Design review of the part built by this model. Coordinates are the model's own, in mm. A direction names the side the tool comes from. Coordinates: 2 decimals unless noted, no trailing zeros. Loops run counter-clockwise (first coordinate to the right, second up) from the corner with the lowest first, then second, coordinate; pieces in that order, holes last.
Q1. Wall thickness on probe 1 along X at (y, z) = (0, 2); probe 2 along Z at (x, y) = (15, 5.5); probe 3 along Z at (x, y) = (-7, 5.75): over which ranges is each line inside the solid? List them lowest first.
Q2. Add section D-D on x = 23. Give the boundary of the cut face in (y, z).
Q3. Add section C-C on x = 15. Give the boundary of the cut face in (y, z), and give its area (4 significant figures).
Q4. For P1, Ø5, axis at x = -12.5, y = -5, coming from the -Z side; P2, Ø3, axis at x = -13, z = 1, coming from the +Y side; P3, Ø7, axis at y = 1.5, z = -20.5, coming from the -X side, all flat-tipped, find the tip position at first contact; note any pin that passes through.
Q5. Add section B-B on y = 0. Give the boundary of the cut face in (x, z), and give its area (3 significant figures).
Q6. Draft analysis for pull direction X (two halves, no side actions). For faces 4 (the face through (25, 0, -25)), 5 (the face through (-12.253, -2.908, -0.121)), 6 (the face through (14, -7, -5)), state which applies: released by +X, released by -X, zero draft, split by the parting line, or undercut.
Q7. Add section A-A on z = 0. Give the boundary of the cut face in (x, y), and give its area (3 significant figures).
Q8. Machinability: for faces 1 (the face through (-25, 0, 0)), 2 (the face through (17.2, 1.3, 2.2)), 3 (the face through (0, 0, -6)), which of the approach directions +Z, -Z, +X, -X, +Y, -Y give a long, thin tool a straight path to every point of the face, cutting with its end or side? Answer none if there is none.
```python
from build123d import *

# Parameters (mm, degrees)
SKETCH1_W                                           = 50
SKETCH1_H                                           = 12
BOSS_EXTRUDE1_DEPTH                                 = 7
HOLE_SIZE_PER_SOCKET_HEAD_CAP_SCREW_TYP_D           = 5.5
HOLE_SIZE_PER_SOCKET_HEAD_CAP_SCREW_TYP_CBORE_D     = 10
HOLE_SIZE_PER_SOCKET_HEAD_CAP_SCREW_TYP_CBORE_DEPTH = 5.7
SKETCH4_W                                           = 15
SKETCH4_H                                           = 40
BOSS_EXTRUDE2_DEPTH                                 = 14
M5_TAPPED_HOLE1_D                                   = 4.2
SKETCH8_R                                           = 2.5
CUT_EXTRUDE1_DEPTH                                  = 55.332310829


with BuildPart() as part:
    # Sketch1 → Boss-Extrude1 (new, symmetric)
    with BuildSketch(Plane(origin=(0, 0, 0), x_dir=(1, 0, 0), z_dir=(0, 1, 0))):
        Rectangle(SKETCH1_W, SKETCH1_H)
    extrude(amount=BOSS_EXTRUDE1_DEPTH, both=True)

    # Hole Size (per socket head cap screw type)1 (through all)
    with Locations(Plane(origin=(0, 7, 0), x_dir=(1, 0, 0), z_dir=(0, 1, 0))):
        with Locations((15, 0), (-15, 0)):
            CounterBoreHole(HOLE_SIZE_PER_SOCKET_HEAD_CAP_SCREW_TYP_D / 2, HOLE_SIZE_PER_SOCKET_HEAD_CAP_SCREW_TYP_CBORE_D / 2, HOLE_SIZE_PER_SOCKET_HEAD_CAP_SCREW_TYP_CBORE_DEPTH)

    # Sketch4 → Boss-Extrude2 (add)
    with BuildSketch(Plane(origin=(0, 7, 0), x_dir=(1, 0, 0), z_dir=(0, 1, 0))):
        with Locations((32.5, 14)):
            Rectangle(SKETCH4_W, SKETCH4_H)
    extrude(amount=-BOSS_EXTRUDE2_DEPTH)

    # M5 Tapped Hole1 (through all)
    with Locations(Plane(origin=(40, 0, 0), x_dir=(0, 0, -1), z_dir=(1, 0, 0))):
        with Locations((21, 0)):
            Hole(M5_TAPPED_HOLE1_D / 2)

    # Sketch8 → Cut-Extrude1 (cut, through all)
    with BuildSketch(Plane(origin=(0, 7, 0), x_dir=(1, 0, 0), z_dir=(0, 1, 0))):
        with Locations((25, 8.5)):
            Circle(SKETCH8_R)
    extrude(amount=-CUT_EXTRUDE1_DEPTH, mode=Mode.SUBTRACT)


solid = part.part
```
Entries:
1. probe 1: x = -25 to -16.89, -13.11 to 13.11, 16.89 to 40
1. probe 2: z = -6 to -5, 5 to 6
1. probe 3: z = -6 to 6
2. outline: (-7, -6) - (7, -6) - (7, 6) - (-7, 6) - close
3. outline: (-7, -6) - (7, -6) - (7, -5) - (1.3, -5) - (1.3, -2.75) - (-7, -2.75) - close; (-7, 2.75) - (1.3, 2.75) - (1.3, 5) - (7, 5) - (7, 6) - (-7, 6) - close
3. area: 65.35 mm2
4. P1: stops at z = -6
4. P2: stops at y = 1.3
4. P3: stops at x = 25
5. outline: (-25, -6) - (25, -6) arc R2.5 cw to (25, -11) - (25, -18.9) - (40, -18.9) - (40, 6) - (-25, 6) - close; (25, -34) - (40, -34) - (40, -23.1) - (25, -23.1) - close; hole circle Ø5.5 at (-15, 0); hole circle Ø5.5 at (15, 0)
5. area: 1,080 mm2
6. face 4: released by -X
6. face 5: undercut
6. face 6: zero draft
7. outline: (-25, -7) - (-17.75, -7) - (-17.75, 1.3) - (-20, 1.3) - (-20, 7) - (-25, 7) - close; (-12.25, -7) - (12.25, -7) - (12.25, 1.3) - (10, 1.3) - (10, 7) - (-10, 7) - (-10, 1.3) - (-12.25, 1.3) - close; (17.75, -7) - (40, -7) - (40, 7) - (20, 7) - (20, 1.3) - (17.75, 1.3) - close
7. area: 705 mm2
8. face 1: +Z, -Z, -X, +Y, -Y
8. face 2: +Y
8. face 3: -Z, -X, +Y, -Y
